Can you work these out from the model? Positions are in its coordinate system, mm. A direction names the side the tool comes from. Coordinates: 2 decimals unless noted, no trailing zeros. Write each loop counter-clockwise with the first axis right and the second up, starting at its lowest first coordinate (ties: lowest second). Pieces come first, ordered by that corner, then holes. Notation, with made-up numbers: (53.5, 81.5) - (109.5, 81.5) arc R35 ccw to (109.5, 119.5) - close; hole circle Ø4 at (-26, 10.5). An arc over 180 degrees is marked (long way). Use one line per item in the form item = value. Start each with the question number.
(1) If we section it at B-B on z = -156: Please give me the cut outline in (x, y).
(2) Thinking about a two-plate mould opening in X: for faces 3 (the face through (350, 15, -207)), 4 (the face through (0, 15, -207)), 5 (the face through (149, 15, -207)), 6 (the face through (12, 15, -207)), which applies, pulls with the +X half, pulls with the -X half, needs draft (parallel to the pull), parting line crosses it, or undercut?
(3) If I drill on probe 1 along X at (y, z) = (15, -64); probe 2 along X at (y, z) = (22.25, -203); probe 3 along Z at (x, y) = (308, 15), over which ranges is the centre line in solid material (lowest first)? Write a range as from..to.
(4) If we section it at D-D on y = 7.75: Please give me the cut outline in (x, z).
(5) If we section it at A-A on x = 186: Please give me the cut outline in (y, z).
(6) If we section it at C-C on x = 39: Please give me the cut outline in (y, z).
(7) On a 3-axis mill with a long thin cutter (end or side, diameter ignored), from which of +Z, -Z, +X, -X, +Y, -Y can I reach the whole of each face in a straight line? I mean faces 1 (the face through (285, 15, -207)), 2 (the face through (211, 30, -213)). Say none if no direction works.
```python
from build123d import *

# Parameters (mm, degrees)
SKETCH1_W           = 350
SKETCH1_H           = 420
SKETCH1_R           = 25
SKETCH1_W_2         = 53
SKETCH1_H_2         = 120
BOSS_EXTRUDE1_DEPTH = 30


with BuildPart() as part:
    # Sketch1 → Boss-Extrude1 (new body)
    with BuildSketch(Plane(origin=(0, 0, 0), x_dir=(1, 0, 0), z_dir=(0, 1, 0))):
        with Locations((175, 210)):
            Rectangle(SKETCH1_W, SKETCH1_H)
        with Locations(Location((311, 64, 0), (0, 0, 270))):
            Circle(SKETCH1_R, mode=Mode.SUBTRACT)
        with Locations(Location((39, 64, 0), (0, 0, 270))):
            Circle(SKETCH1_R, mode=Mode.SUBTRACT)
        with Locations((175.5, 208)):
            Rectangle(SKETCH1_W_2, SKETCH1_H_2, mode=Mode.SUBTRACT)
        with Locations((311.5, 208)):
            Rectangle(SKETCH1_W_2, SKETCH1_H_2, mode=Mode.SUBTRACT)
        with Locations((38.5, 208)):
            Rectangle(SKETCH1_W_2, SKETCH1_H_2, mode=Mode.SUBTRACT)
    extrude(amount=BOSS_EXTRUDE1_DEPTH)


solid = part.part
```
Reported:
q1.outline = (0, 0) - (12, 0) - (12, 30) - (0, 30) - close; (65, 0) - (149, 0) - (149, 30) - (65, 30) - close; (202, 0) - (285, 0) - (285, 30) - (202, 30) - close; (338, 0) - (350, 0) - (350, 30) - (338, 30) - close
q2.face_3 = pulls with the +X half
q2.face_4 = pulls with the -X half
q2.face_5 = undercut
q2.face_6 = undercut
q3.probe_1 = 0..14, 64..286, 336..350
q3.probe_2 = 0..12, 65..149, 202..285, 338..350
q3.probe_3 = -420..-268, -148..-88.82, -39.18..0
q4.outline = (0, -420) - (350, -420) - (350, 0) - (0, 0) - close; hole (12, -268) - (65, -268) - (65, -148) - (12, -148) - close; hole circle Ø50 at (39, -64); hole (149, -268) - (202, -268) - (202, -148) - (149, -148) - close; hole (285, -268) - (338, -268) - (338, -148) - (285, -148) - close; hole circle Ø50 at (311, -64)
q5.outline = (0, -420) - (30, -420) - (30, -268) - (0, -268) - close; (0, -148) - (30, -148) - (30, 0) - (0, 0) - close
q6.outline = (0, -420) - (30, -420) - (30, -268) - (0, -268) - close; (0, -148) - (30, -148) - (30, -89) - (0, -89) - close; (0, -39) - (30, -39) - (30, 0) - (0, 0) - close
q7.face_1 = +Y, -Y
q7.face_2 = +Z, -Z, +X, -X, +Y
